from build123d import *
from OCP.BRepFilletAPI import BRepFilletAPI_MakeChamfer

# Parameters (mm, degrees)
SKETCH_1_W      = 10
SKETCH_1_H      = 60
EXTRUDE_1_DEPTH = 4
CHAMFER_1_SIZE  = 2
CHAMFER_1_SIZE2 = 3.464101615
CHAMFER_2_SIZE  = 1


with BuildPart() as part:
    # 草图1 → 凸台-拉伸1 (new body)
    with BuildSketch(Plane(origin=(0, 0, 0), x_dir=(0, 0, -1), z_dir=(1, 0, 0))):
        Rectangle(SKETCH_1_W, SKETCH_1_H)
    extrude(amount=EXTRUDE_1_DEPTH)

    # 倒角1: one chamfer whose edges measure the first distance from different faces: ONE call of the kernel's chamfer builder (chamfer() names one face for all edges)
    chamfer_1_edges_1 = [part.edges().sort_by_distance(p)[0] for p in [
        (4, 30, 0),
    ]]
    chamfer_1_side_1 = [part.faces().sort_by_distance(p)[0] for p in [
        (2, 30, 0),
    ]]
    chamfer_1_edges_2 = [part.edges().sort_by_distance(p)[0] for p in [
        (4, -30, 0),
    ]]
    chamfer_1_side_2 = [part.faces().sort_by_distance(p)[0] for p in [
        (2, -30, 0),
    ]]
    chamfer_1 = BRepFilletAPI_MakeChamfer(part.part.solid().wrapped)
    for e in chamfer_1_edges_1:
        chamfer_1.Add(CHAMFER_1_SIZE, CHAMFER_1_SIZE2, e.wrapped, chamfer_1_side_1[0].wrapped)  # the first distance lies on this face
    for e in chamfer_1_edges_2:
        chamfer_1.Add(CHAMFER_1_SIZE, CHAMFER_1_SIZE2, e.wrapped, chamfer_1_side_2[0].wrapped)  # the first distance lies on this face
    add(Compound.cast(chamfer_1.Shape()), mode=Mode.REPLACE)

    # 倒角2
    chamfer_2_edges = [part.edges().sort_by_distance(p)[0] for p in [
        (4, 0, 5),
        (4, 0, -5),
    ]]
    chamfer(chamfer_2_edges, length=CHAMFER_2_SIZE)


solid = part.part
Source: CAD feature listing. Evaluate the final solid. Frame: model axes, mm. Coordinates: 2 decimals unless noted, no trailing zeros. Order: outer loops, then holes, each group sorted by start corner. A loop starts at its lowest first (then second) coordinate and runs counter-clockwise, first axis right, second up. Notation, with made-up numbers: M 55,82.5 L 111,82.5 A21 ccw 111,103.5 Z; hole C 88,58 d5. An arc over 180 degrees is marked long. Write each question's results on one line, items separated by ' | '. Start each with the question number.
1. Material intervals for L1, parallel to Y at x = 3, z = -4.25; L2, parallel to X at y = 12, z = 4.5; L3, parallel to Y at x = 3.25, z = -0.5, sorted ascending.
2. Section A-A, the plane y = -18.5. Return the cut outline in (x, z), then the cut area to 3 significant figures.
3. Section B-B, the plane z = -3. Return the cut outline in (x, y), then the cut area to 3 significant figures.
Solution:
1) L1: -28.27 to 28.27 | L2: 0 to 3.5 | L3: -27.83 to 27.83
2) outline: M 0,-5 L 3,-5 L 4,-4 L 4,4 L 3,5 L 0,5 Z | area: 39.0 mm²
3) outline: M 0,-30 L 2,-30 L 4,-26.54 L 4,26.54 L 2,30 L 0,30 Z | area: 233 mm²
